For this review, take the finished solid that the model builds, in its own axes (mm). A direction names the side the tool comes from. Give positions to 0.01 mm unless a question says otherwise; leave off trailing zeros. Loops run counter-clockwise (first coordinate to the right, second up) from the corner with the lowest first, then second, coordinate; pieces in that order, holes last.
```python
from build123d import *

# Parameters (mm, degrees)
SKETCH1_W           = 120
SKETCH1_H           = 500
BOSS_EXTRUDE1_DEPTH = 12
CUT_EXTRUDE1_DEPTH  = 12
CHAMFER1_SIZE       = 10


with BuildPart() as part:
    # Sketch1 → Boss-Extrude1 (new body)
    with BuildSketch(Plane.XY):
        Rectangle(SKETCH1_W, SKETCH1_H)
    extrude(amount=BOSS_EXTRUDE1_DEPTH)

    # Sketch2 → Cut-Extrude1 (cut)
    with BuildSketch(Plane.XY.offset(12)):
        with BuildLine():
            Line((-26, 230), (-26, 203))
            ThreePointArc((-26, 203), (-32.5, 196.5), (-39, 203))
            Line((-39, 203), (-39, 230))
            ThreePointArc((-39, 230), (-32.5, 236.5), (-26, 230))
        make_face()
        with BuildLine():
            Line((26, 230), (26, 203))
            ThreePointArc((26, 203), (32.5, 196.5), (39, 203))
            Line((39, 203), (39, 230))
            ThreePointArc((39, 230), (32.5, 236.5), (26, 230))
        make_face()
        with BuildLine():
            Line((26, -230), (26, -203))
            ThreePointArc((26, -203), (32.5, -196.5), (39, -203))
            Line((39, -203), (39, -230))
            ThreePointArc((39, -230), (32.5, -236.5), (26, -230))
        make_face()
        with BuildLine():
            Line((-26, -230), (-26, -203))
            ThreePointArc((-26, -203), (-32.5, -196.5), (-39, -203))
            Line((-39, -203), (-39, -230))
            ThreePointArc((-39, -230), (-32.5, -236.5), (-26, -230))
        make_face()
    extrude(amount=-CUT_EXTRUDE1_DEPTH, mode=Mode.SUBTRACT)

    # Chamfer1
    chamfer1_edges = [part.edges().sort_by_distance(p)[0] for p in [
        (60, -250, 6),
        (-60, -250, 6),
        (-60, 250, 6),
        (60, 250, 6),
    ]]
    chamfer(chamfer1_edges, length=CHAMFER1_SIZE)


solid = part.part
```
Item 1: Take a section at A-A on x = 32.5. Give the boundary of the cut face in (y, z), and give its area (3 significant figures).
Answer:
outline: (-250, 0) - (-236.5, 0) - (-236.5, 12) - (-250, 12) - close; (-196.5, 0) - (196.5, 0) - (196.5, 12) - (-196.5, 12) - close; (236.5, 0) - (250, 0) - (250, 12) - (236.5, 12) - close
area: 5,040 mm2
Item 2: Take a section at B-B on z = 5. Give the boundary of the cut face in (x, y), and give its area (3 significant figures).
Answer:
outline: (-60, -240) - (-50, -250) - (50, -250) - (60, -240) - (60, 240) - (50, 250) - (-50, 250) - (-60, 240) - close; hole (-39, -230) arc R6.5 ccw to (-26, -230) - (-26, -203) arc R6.5 ccw to (-39, -203) - close; hole (-39, 203) arc R6.5 ccw to (-26, 203) - (-26, 230) arc R6.5 ccw to (-39, 230) - close; hole (26, -230) arc R6.5 ccw to (39, -230) - (39, -203) arc R6.5 ccw to (26, -203) - close; hole (26, 203) arc R6.5 ccw to (39, 203) - (39, 230) arc R6.5 ccw to (26, 230) - close
area: 57,900 mm2
Item 3: For L1, parallel to X at y = -228.5, z = 11; L2, parallel to Y at x = 32, z = 10.25; L3, parallel to X at y = -199.5, z = 6.25, list the stretches that pass through material, from the lowest coordinate up.
Answer:
L1: x = -60 to -39, -26 to 26, 39 to 60
L2: y = -250 to -236.48, -196.52 to 196.52, 236.48 to 250
L3: x = -60 to -37.98, -27.02 to 27.02, 37.98 to 60
Item 4: Tool access review of faces 5 (the flat face through (26, -217, 6)), 6 (the flat face through (-1, -250, 6)): name each direction out of +Z, -Z, +X, -X, +Y, -Y from which nothing blocks a thin tool from reaching the whole face with its end or side.
Answer:
face 5: +Z, -Z
face 6: +Z, -Z, +X, -X, -Y
Item 5: The part is to be moulded in two halves that separate along X. For faces 1 (the flat face through (55, 245, 6)), 2 (the flat face through (-55, -245, 6)), 3 (the flat face through (26, 217, 6)), 4 (the flat face through (-39, 216, 6)), say which applies: released by +X, released by -X, zero draft, split by the parting line, or undercut.
Answer:
face 1: released by +X
face 2: released by -X
face 3: undercut
face 4: undercut
